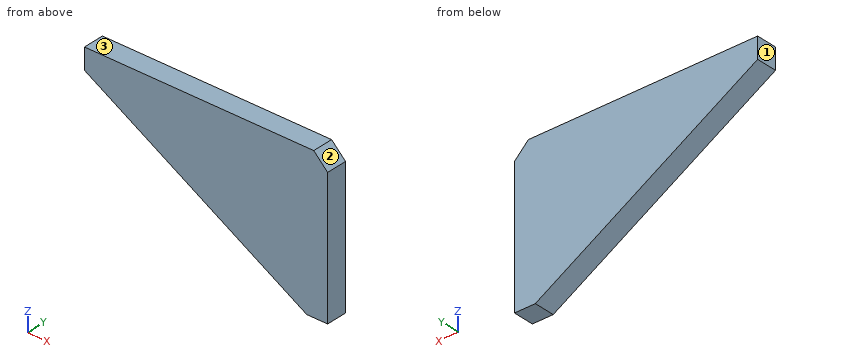
```python
from build123d import *

# Parameters (mm, degrees)
EXTRUDE_1_DEPTH = 30


with BuildPart() as part:
    # 草图1 → 凸台-拉伸1 (new body)
    with BuildSketch(Plane(origin=(0, 0, 0), x_dir=(1, 0, 0), z_dir=(0, 1, 0))):
        Polygon((0, 0), (-30, 0), (-350, -184.752086141), (-350, -214.752086141), (-20, -214.752086141), (0, -194.752086141), align=None)
    extrude(amount=EXTRUDE_1_DEPTH)


solid = part.part
```
Part model, mm, in its own coordinate system. Face numbers are marked on the shaded views. Round coordinates to 2 decimals unless told otherwise and drop trailing zeros. Loops run counter-clockwise (first coordinate to the right, second up) from the corner with the lowest first, then second, coordinate; pieces in that order, holes last.
1. Slice it at B-B (z = 143). Give the cut face in (x, y), and give its area (3 significant figures).
Solutions:
outline: (-277.68, 0) - (0, 0) - (0, 30) - (-277.68, 30) - close
area: 8,330 mm2
2. Slice it at C-C (x = -125). Give the cut face in (y, z), and give its area (3 significant figures).
Solutions:
outline: (0, 54.85) - (30, 54.85) - (30, 214.75) - (0, 214.75) - close
area: 4,800 mm2
3. Flat gauge pins, fed straight in: pin 1 (4 mm diameter, centred on y = 6.5, z = 59, fed in from -X); pin 2 (1 mm diameter, centred on y = 8, z = 39, fed in from +X); pin 3 (8 mm diameter, centred on y = 14.5, z = 130, fed in from -X); pin 4 (10 mm diameter, centred on x = -269, y = 4, fed in from -Z). Where does each tip first touch, or does it go through?
Solutions:
pin 1: stops at x = -135.66
pin 2: stops at x = 0
pin 3: stops at x = -262.09
pin 4: stops at z = 135.1
4. Two-plate mould, pull along X, no slides. Class the marked faces 1, 2 and 3: pulls with the +X half, pulls with the -X half, needs draft (parallel to the pull), parting line crosses it, or undercut.
Solutions:
face 1: pulls with the -X half
face 2: pulls with the +X half
face 3: needs draft
5. Drill centre lines: line 1 along Z through (x, y) = (-197.5, 18); line 2 along X through (y, z) = (16.25, 131); line 3 along Z through (x, y) = (-70, 10.25). Where is each one in solid material? Low to high.
Solutions:
line 1: z = 96.71 to 214.75
line 2: x = -256.9 to 0
line 3: z = 23.09 to 214.75
6. Slice it at A-A (y = 16.5). Give the cut face in (x, z), and give its area (3 significant figures).
Solutions:
outline: (-350, 184.75) - (-30, 0) - (0, 0) - (0, 194.75) - (-20, 214.75) - (-350, 214.75) - close
area: 45,400 mm2
